Input: part model. Units: mm. Frame: model coordinates. A direction names the side the tool comes from. Give positions to 0.01 mm unless a question says otherwise; leave off trailing zeros. Write each loop counter-clockwise with the first axis right and the second up, starting at its lowest first coordinate (ties: lowest second). Pieces come first, ordered by that corner, then holes. Notation, with made-up numbers: (61.25, -34) -> (118.25, -34) arc R27 cw to (118.25, -4) -> close; hole circle Ø10 at (-18.75, -24.5). An arc over 180 degrees is marked (long way). Return JSON: item names as keys, results as strings. Group by question number.
Item 1: Set-up query: faces 1 (the face through (20.572, 44.577, 1225.013)), 2 (the face through (18, 25, 0)). Return all of +Z, -Z, +X, -X, +Y, -Y with unobstructed straight access to the full face (end or side cutting, diameter ignored); none if empty.
Item 2: Section A-A, the plane y = 31. Count the separate pieces of the cut face and the enclosed holes in it, then the cut area to 3 significant figures.
Item 3: Line query: line 1 (X direction, y = 16, z = 50); line 2 (Z direction, x = 52.5, y = 46.5); line 3 (X direction, y = 28, z = 973). Output: solid intervals per line, ascending. Write a range as [from, to].
Item 4: Pin query (flat end, axial travel): P1, Ø13, axis at x = 17.5, z = 1240.5, coming from the +Y side; P2, Ø4, axis at x = 43.5, y = 17.5, coming from the +Z side; P3, Ø20, axis at y = 36, z = 141, coming from the +X side. Return the tip coordinate at first contact, or that it passes through.
Item 5: Section B-B, the plane z = 112.5. Return loops of the section in (x, y), then the cut area to 4 significant figures.
Item 6: Mould query, pull axis X, two halves, no side actions, for faces 3 (the face through (36, 30, 1115)), 4 (the face through (14, 39, 438)), 5 (the face through (47, 35, 938)), 6 (the face through (0, 25, 635)). Classes: released by +X, released by -X, zero draft, split by the parting line, or undercut.
from build123d import *

# Parameters (mm, degrees)
EXTRUDE_1_DEPTH     = 1288
SKETCH_2_R          = 8
CUT_EXTRUDE_1_DEPTH = 725
SKETCH_3_R          = 13
CUT_EXTRUDE_2_DEPTH = 11
CUT_EXTRUDE_3_DEPTH = 350


with BuildPart() as part:
    # 草图1 → 凸台-拉伸1 (new body)
    with BuildSketch(Plane.XY):
        Polygon((0, 0), (0, 50), (64, 50), (29, 0), align=None)
    extrude(amount=EXTRUDE_1_DEPTH)

    # 草图2 → 切除-拉伸1 (cut)
    with BuildSketch(Plane(origin=(0, 50, 0), x_dir=(1, 0, 0), z_dir=(0, 1, 0))):
        with Locations(Location((20, -50, 0), (0, 0, 270))):
            Circle(SKETCH_2_R)
        with Locations(Location((20, -200, 0), (0, 0, 270))):
            Circle(SKETCH_2_R)
        with Locations(Location((20, -444, 0), (0, 0, 270))):
            Circle(SKETCH_2_R)
        with Locations(Location((20, -594, 0), (0, 0, 270))):
            Circle(SKETCH_2_R)
        with Locations(Location((20, -694, 0), (0, 0, 270))):
            Circle(SKETCH_2_R)
        with Locations(Location((20, -844, 0), (0, 0, 270))):
            Circle(SKETCH_2_R)
        with Locations(Location((20, -1088, 0), (0, 0, 270))):
            Circle(SKETCH_2_R)
        with Locations(Location((20, -1238, 0), (0, 0, 270))):
            Circle(SKETCH_2_R)
    extrude(amount=-CUT_EXTRUDE_1_DEPTH, mode=Mode.SUBTRACT)

    # 草图3 → 切除-拉伸2 (cut)
    with BuildSketch(Plane(origin=(0, 50, 0), x_dir=(1, 0, 0), z_dir=(0, 1, 0))):
        with Locations(Location((20, -50, 0), (0, 0, 270))):
            Circle(SKETCH_3_R)
        with Locations(Location((20, -200, 0), (0, 0, 270))):
            Circle(SKETCH_3_R)
        with Locations(Location((20, -444, 0), (0, 0, 270))):
            Circle(SKETCH_3_R)
        with Locations(Location((20, -594, 0), (0, 0, 270))):
            Circle(SKETCH_3_R)
        with Locations(Location((20, -694, 0), (0, 0, 270))):
            Circle(SKETCH_3_R)
        with Locations(Location((20, -844, 0), (0, 0, 270))):
            Circle(SKETCH_3_R)
        with Locations(Location((20, -1088, 0), (0, 0, 270))):
            Circle(SKETCH_3_R)
        with Locations(Location((20, -1238, 0), (0, 0, 270))):
            Circle(SKETCH_3_R)
    extrude(amount=-CUT_EXTRUDE_2_DEPTH, mode=Mode.SUBTRACT)

    # 草图4 → 切除-拉伸3 (cut)
    with BuildSketch(Plane.XY.offset(1288)):
        Polygon((64, 50), (36, 50), (36, 10), align=None)
    cut_extrude_3 = extrude(amount=-CUT_EXTRUDE_3_DEPTH, mode=Mode.SUBTRACT)

    # 镜向1: 切除-拉伸3 across plane
    add(cut_extrude_3.mirror(Plane(origin=(0, 0, 644), x_dir=(1, 0, 0), z_dir=(0, 0, -1))), mode=Mode.SUBTRACT)


solid = part.part
Answer below:
{
 "1": {"face 1": "+Y", "face 2": "-Z, +X, -X, +Y, -Y"},
 "2": {"separate pieces": "1", "enclosed holes": "8", "area": "53,400 mm2"},
 "3": {"line 1": "x = [0, 12], [28, 36]", "line 2": "z = [350, 938]", "line 3": "x = [0, 36]"},
 "4": {"P1": "stops at y = 39", "P2": "stops at z = 938", "P3": "stops at x = 36"},
 "5": {"outline": "(0, 0) -> (29, 0) -> (36, 10) -> (36, 50) -> (0, 50) -> close", "area": "1,765 mm2"},
 "6": {"face 3": "released by +X", "face 4": "undercut", "face 5": "zero draft", "face 6": "released by -X"}
}
